Part model, mm, in its own coordinate system. Face numbers are marked on the shaded views. A direction names the side the tool comes from. Give positions to 0.01 mm unless a question says otherwise; leave off trailing zeros. Write each loop counter-clockwise with the first axis right and the second up, starting at its lowest first coordinate (ties: lowest second). Pieces come first, ordered by that corner, then holes.
from build123d import *

# Parameters (mm, degrees)
BOSS_EXTRUDE1_DEPTH     = 11.43
SKETCH2_R               = 9.525
BOSS_EXTRUDE2_DEPTH     = 11.43
SKETCH8_R               = 3.81
CUT_EXTRUDE6_DEPTH      = 37.167138399
SKETCH9_R               = 3.81
CUT_EXTRUDE7_DEPTH      = 37.167138399
F_1_2_13_TAPPED_HOLE1_D = 10.71626
SKETCH12_W              = 25.4
SKETCH12_H              = 5.08
CUT_EXTRUDE8_DEPTH      = 33.602164039
CIRPATTERN1_COUNT       = 4
FILLET1_R               = 3.81
SCALE1_SCALE            = 2


with BuildPart() as part:
    # Sketch1 → Boss-Extrude1 (new body)
    with BuildSketch(Plane(origin=(0, 0, 0), x_dir=(1, 0, 0), z_dir=(0, 1, 0))):
        Polygon((-5.08, 21.59), (5.08, 21.59), (5.08, 5.08), (21.59, 5.08), (21.59, -5.08), (5.08, -5.08), (5.08, -21.59), (-5.08, -21.59), (-5.08, -5.08), (-21.59, -5.08), (-21.59, 5.08), (-5.08, 5.08), align=None)
    extrude(amount=BOSS_EXTRUDE1_DEPTH)

    # Sketch2 → Boss-Extrude2 (add)
    with BuildSketch(Plane(origin=(0, 11.43, 0), x_dir=(1, 0, 0), z_dir=(0, 1, 0))):
        Circle(SKETCH2_R)
    extrude(amount=-BOSS_EXTRUDE2_DEPTH)

    # Sketch8 → Cut-Extrude6 (cut, through all)
    with BuildSketch(Plane.ZY.offset(5.08)):
        with Locations((14.823623369, 5.715)):
            Circle(SKETCH8_R)
        with Locations((-14.823623369, 5.715)):
            Circle(SKETCH8_R)
    extrude(amount=-CUT_EXTRUDE6_DEPTH, mode=Mode.SUBTRACT)

    # Sketch9 → Cut-Extrude7 (cut, through all)
    with BuildSketch(Plane(origin=(0, 0, -5.08), x_dir=(-1, 0, 0), z_dir=(0, 0, -1))):
        with Locations((14.823623369, 5.715)):
            Circle(SKETCH9_R)
        with Locations((-14.823623369, 5.715)):
            Circle(SKETCH9_R)
    extrude(amount=-CUT_EXTRUDE7_DEPTH, mode=Mode.SUBTRACT)

    # 1/2-13 Tapped Hole1 (through all)
    with Locations(Plane(origin=(0, 11.43, 0), x_dir=(1, 0, 0), z_dir=(0, 1, 0))):
        with Locations((0, 0)):
            Hole(F_1_2_13_TAPPED_HOLE1_D / 2)

    # Sketch12 → Cut-Extrude8 (cut, through all)
    with BuildSketch(Plane(origin=(0, 11.43, 0), x_dir=(1, 0, 0), z_dir=(0, 1, 0))):
        with Locations((-21.59, 0)):
            Rectangle(SKETCH12_W, SKETCH12_H)
    cut_extrude8 = extrude(amount=-CUT_EXTRUDE8_DEPTH, mode=Mode.SUBTRACT)

    # CirPattern1: Cut-Extrude8 ×4 about axis
    cirpattern1_axis = Axis((0, 0, 0), (0, 1, 0))
    for i in range(1, CIRPATTERN1_COUNT):
        add(cut_extrude8.rotate(cirpattern1_axis, i * 360 / CIRPATTERN1_COUNT), mode=Mode.SUBTRACT)

    # Fillet1
    fillet1_edges = [part.edges().sort_by_distance(p)[0] for p in [
        (-21.59, 0, 3.81),
        (-21.59, 11.43, 3.81),
        (21.59, 0, 3.81),
        (-3.81, 0, 21.59),
        (3.81, 0, 21.59),
        (3.81, 11.43, 21.59),
        (-21.59, 0, -3.81),
        (21.59, 0, -3.81),
        (21.59, 11.43, -3.81),
        (3.81, 0, -21.59),
        (-21.59, 11.43, -3.81),
        (-3.81, 0, -21.59),
        (-3.81, 11.43, -21.59),
        (-3.81, 11.43, 21.59),
        (21.59, 11.43, 3.81),
        (3.81, 11.43, -21.59),
    ]]
    fillet(fillet1_edges, radius=FILLET1_R)


with BuildPart() as part_1:
    # Scale1: scaled about (0, 0, 0)
    add(part.part.scale(SCALE1_SCALE))


solid = part_1.part
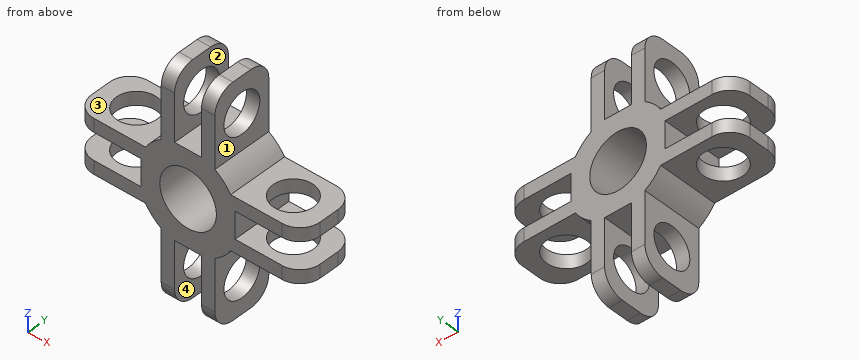
1) Saw through at A-A (z = 0). Write the cut outline in (x, y).
Check result:
outline: (-17.78, 0) - (-10.72, 0) - (-10.72, 22.86) - (-17.78, 22.86) - close; (10.72, 0) - (17.78, 0) - (17.78, 22.86) - (10.72, 22.86) - close
2) Saw through at B-B (x = 0). Write the cut outline in (y, z), and give its area (3 significant figures).
Check result:
outline: (0, -17.78) - (22.86, -17.78) - (22.86, -10.72) - (0, -10.72) - close; (0, 10.72) - (22.86, 10.72) - (22.86, 17.78) - (0, 17.78) - close
area: 323 mm2
3) Flat gauge pins, fed straight in: P1, Ø2, axis at y = 17.5, z = -3.5, coming from the +X side; P2, Ø7, axis at y = 12, z = 30.5, coming from the -X side; P3, Ø11, axis at y = 7, z = -0.5, coming from the +X side; P4, Ø11.5, axis at x = 36, y = 17, coming from the -Z side. Where does each tip first touch, or does it go through?
Check result:
P1: stops at x = 17.78
P2: passes through
P3: stops at x = 43.18
P4: stops at z = -10.16
4) Saw through at D-D (y = 11.43). State how many separate pieces and enclosed holes the cut face has, and give its area (3 significant figures).
Check result:
separate pieces: 9
enclosed holes: 1
area: 1,170 mm2
5) Saw through at C-C (x = 31.5). Write the cut outline in (y, z).
Check result:
outline: (0, -10.16) - (4.04, -10.16) - (4.04, -5.08) - (0, -5.08) - close; (0, 5.08) - (4.04, 5.08) - (4.04, 10.16) - (0, 10.16) - close; (18.82, -10.16) - (22.86, -10.16) - (22.86, -5.08) - (18.82, -5.08) - close; (18.82, 5.08) - (22.86, 5.08) - (22.86, 10.16) - (18.82, 10.16) - close
6) 3-axis set-ups, long thin cutter, end or side, ignore diameter. For the marked faces 1, 2, 3 and 4: which of +Z, -Z, +X, -X, +Y, -Y reach the whole face in a straight line?
Check result:
face 1: +Z, +X, +Y, -Y
face 2: +Z, +Y, -Y
face 3: +Z, -X, +Y, -Y
face 4: -Z, +Y, -Y
7) Drill centre lines: L1, parallel to X at y = 18, z = 0.5; L2, parallel to Z at x = 9, y = 7.75; L3, parallel to Z at x = -37, y = 5. Where is each one in solid material? Low to high.
Check result:
L1: x = -17.78 to -10.7, 10.7 to 17.78
L2: z = -43.18 to -36.32, -22.97 to -5.82, 5.82 to 22.97, 36.32 to 43.18
L3: z = -10.16 to -5.08, 5.08 to 10.16
